The drawing under review shows one solid part. Ordinate dimensions are in mm from its lowest x, y, z. A direction names the side the tool comes from. Round coordinates to 2 decimals unless told otherwise and drop trailing zeros. Write each loop counter-clockwise with the first axis right and the second up, starting at its lowest first coordinate (ties: lowest second). Pieces come first, ordered by that corner, then holes.
Item 1: To check wall thickness, follow L1, parallel to Z at x = 11, y = 1.05; L2, parallel to X at y = 8, z = 1.5; L3, parallel to Y at x = 31, z = 5.25. State the ranges of each line that lie inside material, in increasing order.
Item 2: Add section A-A (z = 4). Give the boundary of the cut face in (x, y), plus the area to 3 significant figures.
Item 3: Add section B-B (y = 3.5). Give the boundary of the cut face in (x, z).
Item 4: Add section C-C (x = 11). Give the boundary of the cut face in (y, z).
Item 5: Draft analysis for pull direction Z (two halves, no side actions). For the marked faces 1, 2 and 3, state which applies: +Z half, -Z half, draft (parallel to the pull), parting line (faces both ways), or undercut.
Item 6: Add section D-D (z = 6.5). Give the boundary of the cut face in (x, y).
Item 7: Clearance check with flat-ended pins moving along their axes: pin 1 Ø2.5 at (y, z) = (10.5, 4) entering from -X; pin 2 Ø4 at (x, z) = (4.5, 5.5) entering from +Y. State where each tip first meets the part, or that it passes through.
Item 8: Machinability: for the marked faces 4, 5 and 6, which of the approach directions +Z, -Z, +X, -X, +Y, -Y give a long, thin tool a straight path to every point of the face, cutting with its end or side? Answer none if there is none.
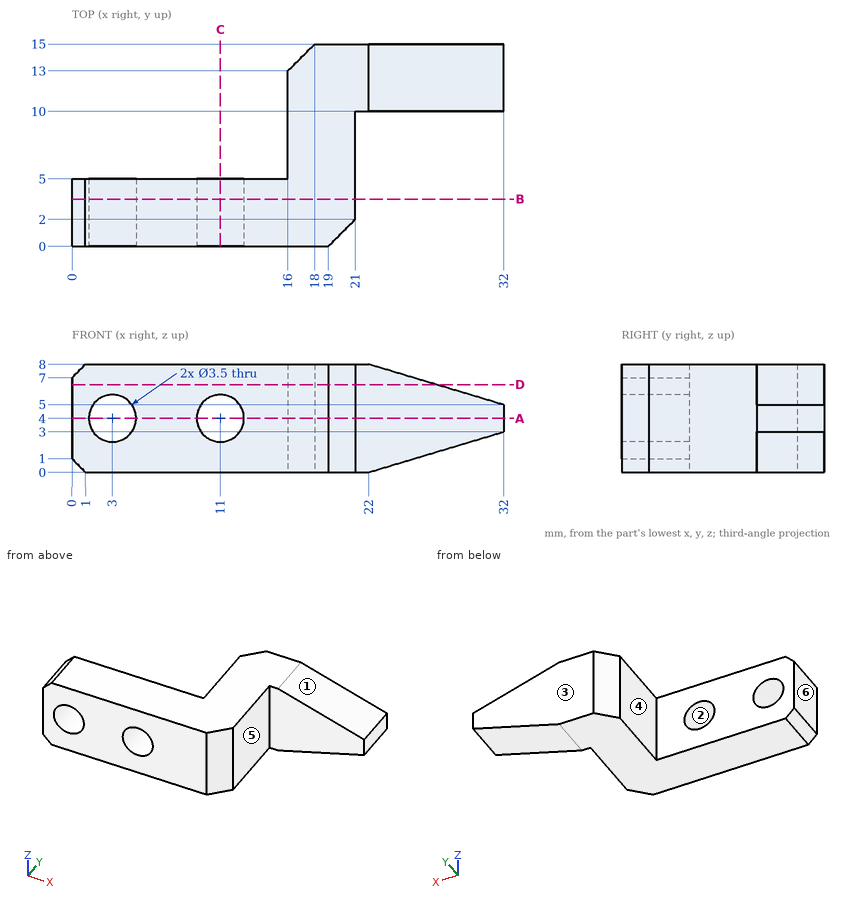
Numbers:
1. L1: z = 0 to 2.25, 5.75 to 8
1. L2: x = 16 to 21
1. L3: y = 10 to 15
2. outline: (0, 0) - (1.25, 0) - (1.25, 5) - (0, 5) - close; (4.75, 0) - (9.25, 0) - (9.25, 5) - (4.75, 5) - close; (12.75, 0) - (19, 0) - (21, 2) - (21, 10) - (32, 10) - (32, 15) - (18, 15) - (16, 13) - (16, 5) - (12.75, 5) - close
2. area: 171 mm2
3. outline: (0, 1) - (1, 0) - (21, 0) - (21, 8) - (1, 8) - (0, 7) - close; hole circle Ø3.5 at (3, 4); hole circle Ø3.5 at (11, 4)
4. outline: (0, 0) - (5, 0) - (5, 2.25) - (0, 2.25) - close; (0, 5.75) - (5, 5.75) - (5, 8) - (0, 8) - close
5. face 1: +Z half
5. face 2: undercut
5. face 3: draft
6. outline: (0, 0) - (19, 0) - (21, 2) - (21, 10) - (27, 10) - (27, 15) - (18, 15) - (16, 13) - (16, 5) - (0, 5) - close
7. pin 1: stops at x = 16
7. pin 2: stops at y = 5
8. face 4: +Z, -Z, -X, +Y
8. face 5: +Z, -Z, +X, -Y
8. face 6: +Z, -Z, -X, +Y, -Y
